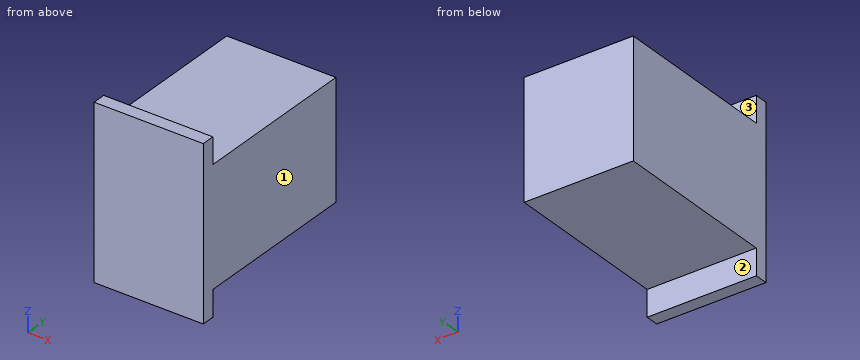
from build123d import *

# Parameters (mm, degrees)
SKETCH1_W           = 50
SKETCH1_H           = 83
BOSS_EXTRUDE1_DEPTH = 39
SKETCH2_W           = 12
SKETCH2_H           = 77
CUT_EXTRUDE1_DEPTH  = 76.784233189


with BuildPart() as part:
    # Sketch1 → Boss-Extrude1 (new, symmetric)
    with BuildSketch(Plane.XY):
        Rectangle(SKETCH1_W, SKETCH1_H)
    extrude(amount=BOSS_EXTRUDE1_DEPTH, both=True)

    # Sketch2 → Cut-Extrude1 (cut, through all)
    with BuildSketch(Plane.ZY.offset(25)):
        with Locations((-33, 3)):
            Rectangle(SKETCH2_W, SKETCH2_H)
        with Locations((33, 3)):
            Rectangle(SKETCH2_W, SKETCH2_H)
    extrude(amount=-CUT_EXTRUDE1_DEPTH, mode=Mode.SUBTRACT)


solid = part.part
Work out the finished part from the listing and answer in its coordinate system (mm). Face numbers are marked on the shaded views. A direction names the side the tool comes from. Round coordinates to 2 decimals unless told otherwise and drop trailing zeros. Loops run counter-clockwise (first coordinate to the right, second up) from the corner with the lowest first, then second, coordinate; pieces in that order, holes last. Notation, with made-up numbers: (-5.75, 16.5) - (15.25, 16.5) arc R21 ccw to (15.25, 45.5) - close; hole circle Ø1 at (50, -14.5). An arc over 180 degrees is marked (long way). One line per item, written item: value.
Q1. Find section B-B on z = -29. Give the vertices of the cut face in (x, y), and give its area (3 significant figures).
Check values:
outline: (-25, -41.5) - (25, -41.5) - (25, -35.5) - (-25, -35.5) - close
area: 300 mm2
Q2. Straight lines are drawn through the part: probe 1 along Z at (x, y) = (-0.5, -10); probe 2 along Y at (x, z) = (9.5, 35). For each, find the intervals that lie inside material, in ascending order.
Check values:
probe 1: -27 to 27
probe 2: -41.5 to -35.5
Q3. Find section A-A on x = 7.5. Give the vertices of the cut face in (y, z), and give its area (3 significant figures).
Check values:
outline: (-41.5, -39) - (-35.5, -39) - (-35.5, -27) - (41.5, -27) - (41.5, 27) - (-35.5, 27) - (-35.5, 39) - (-41.5, 39) - close
area: 4,630 mm2
Q4. Each of these flat-tipped pins is pushed along its axis until it touches: pin 1 Ø25 at (x, y) = (-7, 4.5) entering from +Z; pin 2 Ø4 at (x, y) = (16, -13) entering from -Z. Where does it stop, or does it pass through?
Check values:
pin 1: z = 27
pin 2: z = -27
Q5. Find section C-C on y = 31. Give the vertices of the cut face in (x, z), and give its area (3 significant figures).
Check values:
outline: (-25, -27) - (25, -27) - (25, 27) - (-25, 27) - close
area: 2,700 mm2
Q6. For the marked faces 1, 2 and 3, determine the directions among +Z, -Z, +X, -X, +Y, -Y from which every point of the face is accessible in a straight line to the end or side of a thin tool.
Check values:
face 1: +Z, -Z, +X, +Y, -Y
face 2: -Z, +X, -X, +Y
face 3: +Z, +X, -X, +Y
